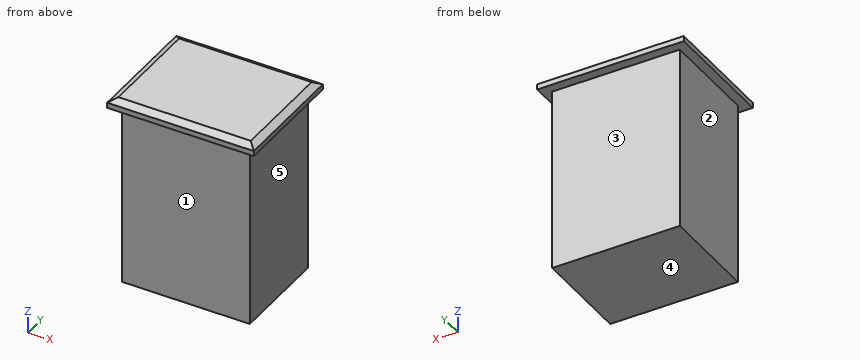
from build123d import *

# Parameters (mm, degrees)
SKETCH1_W           = 27
SKETCH1_H           = 21
BOSS_EXTRUDE1_DEPTH = 39
SKETCH2_W           = 31
SKETCH2_H           = 25
BOSS_EXTRUDE2_DEPTH = 2
CHAMFER1_SIZE       = 1.5
CHAMFER1_SIZE2      = 0.866025404


with BuildPart() as part:
    # Sketch1 → Boss-Extrude1 (new body)
    with BuildSketch(Plane.XY):
        Rectangle(SKETCH1_W, SKETCH1_H)
    extrude(amount=BOSS_EXTRUDE1_DEPTH)

    # Sketch2 → Boss-Extrude2 (add)
    with BuildSketch(Plane.XY.offset(39)):
        Rectangle(SKETCH2_W, SKETCH2_H)
    extrude(amount=BOSS_EXTRUDE2_DEPTH)

    # Chamfer1
    chamfer1_edges = [part.edges().sort_by_distance(p)[0] for p in [
        (15.5, 0, 41),
        (0, 12.5, 41),
        (-15.5, 0, 41),
        (0, -12.5, 41),
    ]]
    chamfer1_side = [part.faces().sort_by_distance(p)[0] for p in [
        (0, 0, 41),
    ]]
    chamfer(chamfer1_edges, length=CHAMFER1_SIZE, length2=CHAMFER1_SIZE2, reference=chamfer1_side[0])


solid = part.part
Geometry check sheet. Reference: the model listing, model coordinates, mm. Face numbers are marked on the shaded views. A direction names the side the tool comes from. Give positions to 0.01 mm unless a question says otherwise; leave off trailing zeros. Order: outer loops, then holes, each group sorted by start corner. A loop starts at its lowest first (then second) coordinate and runs counter-clockwise, first axis right, second up.
1. Access from +Z, -Z, +X, -X, +Y, -Y to the whole of each face (thin tool, end or side, straight path). Record for the marked faces 1, 2, 3, 4 and 5.
Completed:
face 1: -Z, +X, -X, -Y
face 2: -Z, -X, +Y, -Y
face 3: -Z, +X, -X, +Y
face 4: -Z, +X, -X, +Y, -Y
face 5: -Z, +X, +Y, -Y
2. Sectioned sample at A-A (x = 4). Record the boundary of the cut face in (y, z).
Completed:
outline: (-12.5, 39) - (-10.5, 39) - (-10.5, 0) - (10.5, 0) - (10.5, 39) - (12.5, 39) - (12.5, 40.13) - (11, 41) - (-11, 41) - (-12.5, 40.13) - close
3. Depth check by flat-ended pin: pin 1 (3 mm diameter, centred on y = 1, z = 12, fed in from +X); pin 2 (8 mm diameter, centred on x = 4.5, z = 28.5, fed in from +Y); pin 3 (2 mm diameter, centred on y = -3.5, z = 19.5, fed in from -X). Enter the tip coordinate at first touch or a pass-through.
Completed:
pin 1: stops at x = 13.5
pin 2: stops at y = 10.5
pin 3: stops at x = -13.5
4. Sectioned sample at C-C (z = 25). Record the boundary of the cut face in (x, y).
Completed:
outline: (-13.5, -10.5) - (13.5, -10.5) - (13.5, 10.5) - (-13.5, 10.5) - close
5. Sectioned sample at B-B (y = -8). Record the boundary of the cut face in (x, z).
Completed:
outline: (-15.5, 39) - (-13.5, 39) - (-13.5, 0) - (13.5, 0) - (13.5, 39) - (15.5, 39) - (15.5, 40.13) - (14, 41) - (-14, 41) - (-15.5, 40.13) - close
6. Scan lines: line 1 (X direction, y = 9.5, z = 3); line 2 (Y direction, x = 11.5, z = 36.5). Record each from-to range of solid material in increasing order.
Completed:
line 1: x = -13.5 to 13.5
line 2: y = -10.5 to 10.5
